```python
from build123d import *

# Parameters (mm, degrees)
SKETCH_1_R      = 40
SKETCH_1_R_2    = 4.5
EXTRUDE_1_DEPTH = 1.5


with BuildPart() as part:
    # 草图1 → 凸台-拉伸1 (new body)
    with BuildSketch(Plane.XY):
        with BuildLine():
            ThreePointArc((15.612494996, -47.5), (35.355339059, -35.355339059), (47.5, -15.612494996))
            ThreePointArc((47.5, -15.612494996), (49.788897449, -11.806790765), (53.5, -9.367496998))
            ThreePointArc((53.5, -9.367496998), (60, 0), (53.5, 9.367496998))
            ThreePointArc((53.5, 9.367496998), (49.788897449, 11.806790765), (47.5, 15.612494996))
            ThreePointArc((47.5, 15.612494996), (35.355339059, 35.355339059), (15.612494996, 47.5))
            ThreePointArc((15.612494996, 47.5), (11.806790765, 49.788897449), (9.367496998, 53.5))
            ThreePointArc((9.367496998, 53.5), (0, 60), (-9.367496998, 53.5))
            ThreePointArc((-9.367496998, 53.5), (-11.806790765, 49.788897449), (-15.612494996, 47.5))
            ThreePointArc((-15.612494996, 47.5), (-35.355339059, 35.355339059), (-47.5, 15.612494996))
            ThreePointArc((-47.5, 15.612494996), (-49.788897449, 11.806790765), (-53.5, 9.367496998))
            ThreePointArc((-53.5, 9.367496998), (-60, 0), (-53.5, -9.367496998))
            ThreePointArc((-53.5, -9.367496998), (-49.788897449, -11.806790765), (-47.5, -15.612494996))
            ThreePointArc((-47.5, -15.612494996), (-35.355339059, -35.355339059), (-15.612494996, -47.5))
            ThreePointArc((-15.612494996, -47.5), (-11.806790765, -49.788897449), (-9.367496998, -53.5))
            ThreePointArc((-9.367496998, -53.5), (0, -60), (9.367496998, -53.5))
            ThreePointArc((9.367496998, -53.5), (11.806790765, -49.788897449), (15.612494996, -47.5))
        make_face()
        Circle(SKETCH_1_R, mode=Mode.SUBTRACT)
        with Locations((0, 50)):
            Circle(SKETCH_1_R_2, mode=Mode.SUBTRACT)
        with Locations((-50, 0)):
            Circle(SKETCH_1_R_2, mode=Mode.SUBTRACT)
        with Locations((0, -50)):
            Circle(SKETCH_1_R_2, mode=Mode.SUBTRACT)
        with Locations((50, 0)):
            Circle(SKETCH_1_R_2, mode=Mode.SUBTRACT)
    extrude(amount=EXTRUDE_1_DEPTH)


solid = part.part
```
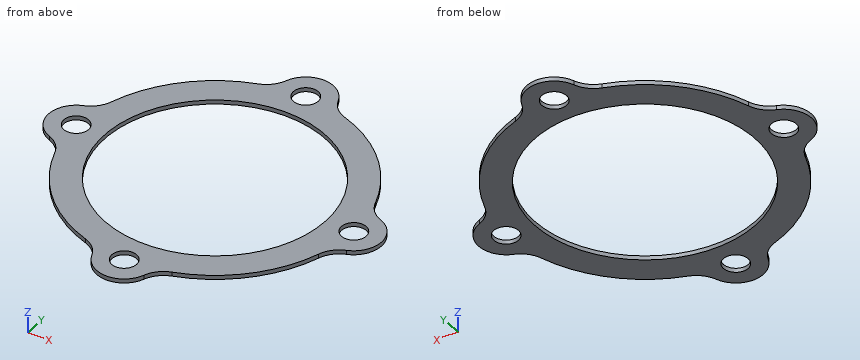
The listing builds one solid part. Answer for the finished solid, in the listing's coordinates (mm). Coordinates: 2 decimals unless noted, no trailing zeros. Loops run counter-clockwise (first coordinate to the right, second up) from the corner with the lowest first, then second, coordinate; pieces in that order, holes last. Notation, with made-up numbers: (67.5, 37.25) - (77.5, 37.25) arc R31 ccw to (77.5, 62.25) - close; hole circle Ø9 at (-23.5, 30.25). An arc over 180 degrees is marked (long way). Use a Markdown table: item, result. Add a question column.
1) Given pin 1 (8 mm diameter, centred on x = -50, y = 0, fed in from -Z), flat-ended and moving along its own axis, determine where the tip first touches the part or whether it passes through.
2) The part is cut by section C-C, the plane y = 50. Give the vertices of the cut face in (x, z).
3) The part is cut by section A-A, the plane x = 0. Give the vertices of the cut face in (y, z), and give its area (3 significant figures).
4) Find the intervals of material crossed by line 1 (Y direction, x = 0, z = 0.9); line 2 (X direction, y = 4, z = 1.25); line 3 (Y direction, x = 7, z = 0.8), in increasing order.
5) The part is cut by section B-B, the plane z = 0.8. Give the vertices of the cut face in (x, y) (1 decimal), and give its area (3 significant figures).
Here are the results:
| question | item | result |
|---|---|---|
| 1 | pin 1 | passes through |
| 2 | outline | (-11.59, 0) - (-4.5, 0) - (-4.5, 1.5) - (-11.59, 1.5) - close; (4.5, 0) - (11.59, 0) - (11.59, 1.5) - (4.5, 1.5) - close |
| 3 | outline | (-60, 0) - (-54.5, 0) - (-54.5, 1.5) - (-60, 1.5) - close; (-45.5, 0) - (-40, 0) - (-40, 1.5) - (-45.5, 1.5) - close; (40, 0) - (45.5, 0) - (45.5, 1.5) - (40, 1.5) - close; (54.5, 0) - (60, 0) - (60, 1.5) - (54.5, 1.5) - close |
| 3 | area | 33.0 mm^2 |
| 4 | line 1 | y = -60 to -54.5, -45.5 to -40, 40 to 45.5, 54.5 to 60 |
| 4 | line 2 | x = -59.17 to -52.06, -47.94 to -39.8, 39.8 to 47.94, 52.06 to 59.17 |
| 4 | line 3 | y = -57.14 to -39.38, 39.38 to 57.14 |
| 5 | outline | (-53.5, -9.4) arc R10 cw to (-47.5, -15.6) arc R50 ccw to (-15.6, -47.5) arc R10 cw to (-9.4, -53.5) arc R10 ccw to (9.4, -53.5) arc R10 cw to (15.6, -47.5) arc R50 ccw to (47.5, -15.6) arc R10 cw to (53.5, -9.4) arc R10 ccw to (53.5, 9.4) arc R10 cw to (47.5, 15.6) arc R50 ccw to (15.6, 47.5) arc R10 cw to (9.4, 53.5) arc R10 ccw to (-9.4, 53.5) arc R10 cw to (-15.6, 47.5) arc R50 ccw to (-47.5, 15.6) arc R10 cw to (-53.5, 9.4) arc R10 ccw to start; hole circle Ø9 at (-50, 0); hole circle Ø80 at (0, 0); hole circle Ø9 at (0, -50); hole circle Ø9 at (0, 50); hole circle Ø9 at (50, 0) |
| 5 | area | 3,270 mm^2 |
